from build123d import *

# Parameters (mm, degrees)
EXTRUDE_1_DEPTH        = 12
HOLE_WIZARD_M6_1_D     = 5
HOLE_WIZARD_M6_1_DEPTH = 15
HOLE_WIZARD_M6_1_TIP   = 1.502151548
HOLE_WIZARD_M6_2_D     = 5
HOLE_WIZARD_M6_2_DEPTH = 15
HOLE_WIZARD_M6_2_TIP   = 1.502151548
HOLE_WIZARD_M6_3_D     = 5
HOLE_WIZARD_M6_3_DEPTH = 15
HOLE_WIZARD_M6_3_TIP   = 1.502151548


with BuildPart() as part:
    # 草图1 → 凸台-拉伸1 (new body)
    with BuildSketch(Plane.XY):
        Polygon((0, 0), (0, -60), (140, -60), (140, -50), (28, 0), align=None)
    extrude(amount=EXTRUDE_1_DEPTH)

    # M6 螺纹孔1
    with Locations(Plane.ZY):
        with Locations((6, -15), (6, -45)):
            Hole(HOLE_WIZARD_M6_1_D / 2, depth=HOLE_WIZARD_M6_1_DEPTH)
            with Locations((0, 0, -(HOLE_WIZARD_M6_1_DEPTH + HOLE_WIZARD_M6_1_TIP / 2))):  # 118° drill point
                Cone(0, HOLE_WIZARD_M6_1_D / 2, HOLE_WIZARD_M6_1_TIP, mode=Mode.SUBTRACT)

    # M6 螺纹孔2
    with Locations(Plane(origin=(0, -60, 0), x_dir=(-1, 0, 0), z_dir=(0, -1, 0))):
        with Locations((-120, -6), (-20, -6)):
            Hole(HOLE_WIZARD_M6_2_D / 2, depth=HOLE_WIZARD_M6_2_DEPTH)
            with Locations((0, 0, -(HOLE_WIZARD_M6_2_DEPTH + HOLE_WIZARD_M6_2_TIP / 2))):  # 118° drill point
                Cone(0, HOLE_WIZARD_M6_2_D / 2, HOLE_WIZARD_M6_2_TIP, mode=Mode.SUBTRACT)

    # M6 螺纹孔3
    with Locations(Plane(origin=(0, 0, 0), x_dir=(1, 0, 0), z_dir=(0, 1, 0))):
        with Locations((20, -6)):
            Hole(HOLE_WIZARD_M6_3_D / 2, depth=HOLE_WIZARD_M6_3_DEPTH)
            with Locations((0, 0, -(HOLE_WIZARD_M6_3_DEPTH + HOLE_WIZARD_M6_3_TIP / 2))):  # 118° drill point
                Cone(0, HOLE_WIZARD_M6_3_D / 2, HOLE_WIZARD_M6_3_TIP, mode=Mode.SUBTRACT)


solid = part.part
Geometry check sheet. Reference: the model listing, model coordinates, mm. A direction names the side the tool comes from. Coordinates: 2 decimals unless noted, no trailing zeros. Write each loop counter-clockwise with the first axis right and the second up, starting at its lowest first coordinate (ties: lowest second). Pieces come first, ordered by that corner, then holes. Notation, with made-up numbers: (18, -2) -> (73, -2) arc R13 cw to (73, 22) -> close; hole circle Ø4 at (67.5, 49). An arc over 180 degrees is marked (long way). One line per question, with ' | ' between items.
1. Depth check by flat-ended pin: pin 1 Ø1 at (y, z) = (-51.5, 8) entering from -X; pin 2 Ø1 at (x, z) = (124, 6) entering from +Y; pin 3 Ø3 at (x, z) = (120, 6) entering from +Y; pin 4 Ø4.5 at (x, z) = (20, 6) entering from -Y. Enter the tip coordinate at first touch or a pass-through.
Answers:
pin 1: stops at x = 0 | pin 2: stops at y = -42.63 | pin 3: stops at y = -40.4 | pin 4: stops at y = -44.85
2. Cross-section at A-A on y = -56. Record the cut outline in (x, z).
Answers:
outline: (0, 0) -> (140, 0) -> (140, 12) -> (0, 12) -> close; hole circle Ø5 at (20, 6); hole circle Ø5 at (120, 6)
3. Cross-section at C-C on y = -31. Record the cut outline in (x, z), and give its area (3 significant figures).
Answers:
outline: (0, 0) -> (97.44, 0) -> (97.44, 12) -> (0, 12) -> close | area: 1,170 mm²
4. Set-up check for faces 5 (the cylindrical face through (22.5, -7.6, 5.9)), 6 (the cylindrical face through (17.5, -52.4, 5.9)), 7 (the flat face through (84.78, -25.35, 5.92)), 8 (the cylindrical face through (7.6, -15.96, 3.69)): record each of +Z, -Z, +X, -X, +Y, -Y from which the full face is reachable in a straight line by a thin tool's end or side.
Answers:
face 5: +Y | face 6: -Y | face 7: +Z, -Z, +X, +Y | face 8: -X
5. Draft check along Z on faces 1 (the flat face through (53, -36, 0)), 2 (the conical face through (19.68, -16.241, 5.707)), 3 (the flat face through (69, -60, 6)), 4 (the conical face through (16.24, -14.57, 5.94)). Enter one of: +Z half, -Z half, draft (parallel to the pull), parting line (faces both ways), or undercut.
Answers:
face 1: -Z half | face 2: undercut | face 3: draft | face 4: undercut
6. Thickness scan on probe 1 along Y at (x, z) = (9.5, 6); probe 2 along Z at (x, y) = (120, -50.75); probe 3 along Y at (x, z) = (8, 4.25). Record the ranges inside material, lowest first. Write a range as from..to.
Answers:
probe 1: y = -60..-47.5, -42.5..-17.5, -12.5..0 | probe 2: z = 0..3.5, 8.5..12 | probe 3: y = -60..-46.79, -43.21..-16.79, -13.21..0
7. Cross-section at B-B on x = 101. Record the cut outline in (y, z).
Answers:
outline: (-60, 0) -> (-32.59, 0) -> (-32.59, 12) -> (-60, 12) -> close
